```python
from build123d import *

# Parameters (mm, degrees)
SKETCH1_R           = 1
BOSS_EXTRUDE1_DEPTH = 1
SKETCH2_W           = 4
SKETCH2_H           = 11
BOSS_EXTRUDE2_DEPTH = 3
SKETCH3_W           = 3
SKETCH3_H           = 11
CUT_EXTRUDE1_DEPTH  = 10
SKETCH4_W           = 0.703476056
SKETCH4_H           = 9.036961638
CUT_EXTRUDE2_DEPTH  = 3
SKETCH5_W           = 0.607326988
SKETCH5_H           = 8.712280381
BOSS_EXTRUDE3_DEPTH = 4


with BuildPart() as part:
    # Sketch1 → Boss-Extrude1 (new body)
    with BuildSketch(Plane.XY):
        Polygon((-5, 10), (5, 10), (5, 5.5), (9, 5.5), (9, -5.5), (5, -5.5), (5, -10), (-5, -10), align=None)
        with Locations((0, 7)):
            Circle(SKETCH1_R, mode=Mode.SUBTRACT)
        with Locations((0, -7)):
            Circle(SKETCH1_R, mode=Mode.SUBTRACT)
    extrude(amount=BOSS_EXTRUDE1_DEPTH)

    # Sketch2 → Boss-Extrude2 (add)
    with BuildSketch(Plane.XY.offset(1)):
        with Locations((7, 0)):
            Rectangle(SKETCH2_W, SKETCH2_H)
    extrude(amount=BOSS_EXTRUDE2_DEPTH)

    # Sketch3 → Cut-Extrude1 (cut)
    with BuildSketch(Plane(origin=(9, 0, 0), x_dir=(0, 0, -1), z_dir=(1, 0, 0))):
        with Locations((-2.5, 0)):
            Rectangle(SKETCH3_W, SKETCH3_H)
        with BuildLine():
            Line((-1.303663494, 4.247913105), (-1.303663494, -4.13968602))
            ThreePointArc((-1.303663494, -4.13968602), (-2.5, -5.336022526), (-3.696336506, -4.13968602))
            Line((-3.696336506, -4.13968602), (-3.696336506, 4.247913105))
            ThreePointArc((-3.696336506, 4.247913105), (-2.5, 5.444249611), (-1.303663494, 4.247913105))
        make_face(mode=Mode.SUBTRACT)
    extrude(amount=-CUT_EXTRUDE1_DEPTH, mode=Mode.SUBTRACT)


with BuildPart() as cut_extrude1_piece_1:
    # of the separate pieces the step leaves, piece 1, a body of its own (cut_extrude1_pieces)
    add(part.part.solids().sort_by_distance((-5, 10, 0))[0])



with BuildPart() as cut_extrude1_piece_2:
    # of the separate pieces the step leaves, piece 2, a body of its own (cut_extrude1_pieces)
    add(part.part.solids().sort_by_distance((9, 4.247913105, 3.696336506))[0])

    # Sketch4 → Cut-Extrude2 (cut)
    with BuildSketch(Plane(origin=(9, 0, 0), x_dir=(0, 0, -1), z_dir=(1, 0, 0))):
        with Locations((-2.456945609, 0.054113543)):
            Rectangle(SKETCH4_W, SKETCH4_H)
    extrude(amount=-CUT_EXTRUDE2_DEPTH, mode=Mode.SUBTRACT)


with BuildPart() as cut_extrude1_piece_1_1:
    add(cut_extrude1_piece_1.part)

    add(cut_extrude1_piece_2.part)  # Boss-Extrude3 merges Cut-Extrude1 piece 2
    # Sketch5 → Boss-Extrude3 (add)
    with BuildSketch(Plane(origin=(9, 0, 0), x_dir=(0, 0, -1), z_dir=(1, 0, 0))):
        with Locations((-1.303663494, 0.054113543)):
            Rectangle(SKETCH5_W, SKETCH5_H)
    extrude(amount=-BOSS_EXTRUDE3_DEPTH)


solid = cut_extrude1_piece_1_1.part
```
CAD build for the part. Positions are in the model's coordinates, mm. A direction names the side the tool comes from. Round coordinates to 2 decimals unless told otherwise and drop trailing zeros. Write each loop counter-clockwise with the first axis right and the second up, starting at its lowest first coordinate (ties: lowest second). Pieces come first, ordered by that corner, then holes. Notation, with made-up numbers: (45, -11.5) -> (99, -11.5) arc R33 cw to (99, 27.5) -> close; hole circle Ø3 at (-8.75, 24.5). An arc over 180 degrees is marked (long way). Answer in a Markdown table with one row per item. Add a question column.
Item 1: Drill centre lines: line 1 (Y direction, x = 0, z = 0.6); line 2 (Y direction, x = 0.75, z = 0.5); line 3 (X direction, y = 1.5, z = 3.4). Where is each one in solid material? Low to high. Write a range as from..to.
Item 2: Drop flat-ended pins along their axis: pin 1 Ø1.1 at (x, z) = (8, 0.5) entering from -Y; pin 2 Ø1.1 at (y, z) = (-7, 0.5) entering from +X; pin 3 Ø3.5 at (x, y) = (8, -1.5) entering from -Z; pin 4 Ø2 at (x, z) = (7.5, 3) entering from -Y. Give the stop position or say it passes through.
Item 3: Saw through at C-C, the plane y = -7. Write the cut outline in (x, z), then the cut area to 3 significant figures.
Item 4: Saw through at B-B, the plane x = 0. Write the cut outline in (y, z).
Item 5: Saw through at D-D, the plane y = 1. Write the cut outline in (x, z).
Item 6: Which spindle directions (+Z, -Z, +X, -X, +Y, -Y) get a long thin tool onto all of the face, cutting with end or side? Do faces 5 (the face through (7, 5.5, 0.5)), 6 (the face through (-0.13, -6.01, 0.49)), 7 (the face through (7, -5.5, 0.5)), 8 (the face through (5, 0, 2)), 9 (the face through (8, 0, 2.105)). Say none if no direction does.
Item 7: Mould opens along Y. For faces 1 (the face through (9, 0.1, 1.9)), 2 (the face through (0.1, -10, 0.5)), 3 (the face through (-0.1, 10, 0.5)), 4 (the face through (-0.13, 7.99, 0.49)) say: pulls with the +Y half, pulls with the -Y half, needs draft (parallel to the pull), parting line crosses it, or undercut.
Item 8: Saw through at A-A, the plane z = 0.2. Write the cut outline in (x, y), then the cut area to 3 significant figures.
Findings below:
| question | item | result |
|---|---|---|
| 1 | line 1 | y = -10..-8, -6..6, 8..10 |
| 1 | line 2 | y = -10..-7.66, -6.34..6.34, 7.66..10 |
| 1 | line 3 | x = 5..9 |
| 2 | pin 1 | stops at y = -5.5 |
| 2 | pin 2 | stops at x = 5 |
| 2 | pin 3 | stops at z = 0 |
| 2 | pin 4 | stops at y = -5.34 |
| 3 | outline | (-5, 0) -> (-1, 0) -> (-1, 1) -> (-5, 1) -> close; (1, 0) -> (5, 0) -> (5, 1) -> (1, 1) -> close |
| 3 | area | 8.00 mm^2 |
| 4 | outline | (-10, 0) -> (-8, 0) -> (-8, 1) -> (-10, 1) -> close; (-6, 0) -> (6, 0) -> (6, 1) -> (-6, 1) -> close; (8, 0) -> (10, 0) -> (10, 1) -> (8, 1) -> close |
| 5 | outline | (-5, 0) -> (9, 0) -> (9, 2.11) -> (6, 2.11) -> (6, 2.81) -> (9, 2.81) -> (9, 3.7) -> (5, 3.7) -> (5, 1) -> (-5, 1) -> close |
| 6 | face 5 | +Z, -Z, +X, +Y |
| 6 | face 6 | +Z, -Z |
| 6 | face 7 | +Z, -Z, +X, -Y |
| 6 | face 8 | +Z, -X, +Y, -Y |
| 6 | face 9 | +X |
| 7 | face 1 | needs draft |
| 7 | face 2 | pulls with the -Y half |
| 7 | face 3 | pulls with the +Y half |
| 7 | face 4 | undercut |
| 8 | outline | (-5, -10) -> (5, -10) -> (5, -5.5) -> (9, -5.5) -> (9, 5.5) -> (5, 5.5) -> (5, 10) -> (-5, 10) -> close; hole circle Ø2 at (0, -7); hole circle Ø2 at (0, 7) |
| 8 | area | 238 mm^2 |
